Design review of the part shown in the three views and the two pictorial views. Dimensions are in mm from the part's minimum x, y and z. A direction names the side the tool comes from. Round coordinates to 2 decimals unless told otherwise and drop trailing zeros. Loops run counter-clockwise (first coordinate to the right, second up) from the corner with the lowest first, then second, coordinate; pieces in that order, holes last.
1) Take a section at B-B (y = 116). State the section outline as (x, z) points, then the cut area to 3 significant figures.
2) Wall thickness on L1, parallel to Y at x = 194.5, z = 701: over which ranges is the line inside the solid? List them lowest first.
3) Mouldability with a two-part tool opening along X and no side actions: class the marked faces 3, 4 and 5 as pulls with the +X half, pulls with the -X half, needs draft (parallel to the pull), parting line crosses it, or undercut.
4) Take a section at A-A (z = 564.5). State the section outline as (x, y) points.
5) Tool access review of the marked faces 1 and 2: name each direction out of +Z, -Z, +X, -X, +Y, -Y from which nothing blocks a thin tool from reaching the whole face with its end or side.
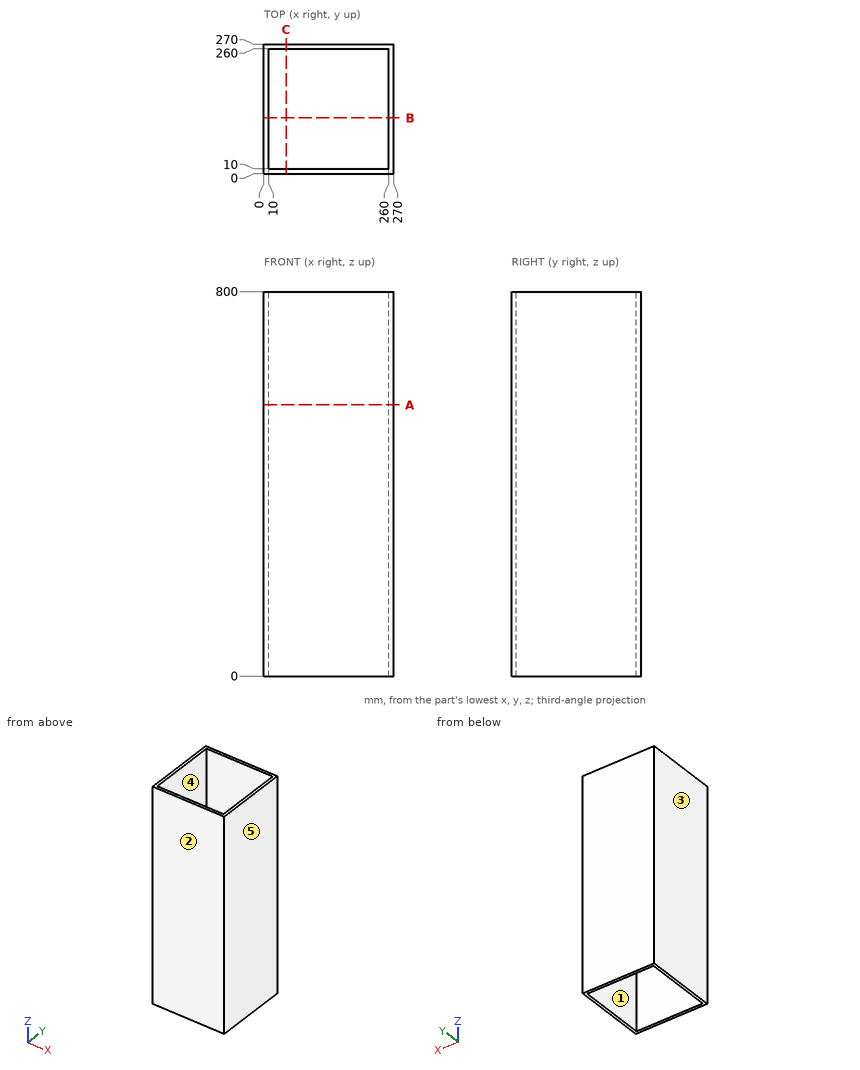
Response:
1. outline: (0, 0) - (10, 0) - (10, 800) - (0, 800) - close; (260, 0) - (270, 0) - (270, 800) - (260, 800) - close
1. area: 16,000 mm2
2. L1: y = 0 to 10, 260 to 270
3. face 3: pulls with the -X half
3. face 4: undercut
3. face 5: pulls with the +X half
4. outline: (0, 0) - (270, 0) - (270, 270) - (0, 270) - close; hole (10, 10) - (260, 10) - (260, 260) - (10, 260) - close
5. face 1: +Z, -Z
5. face 2: +Z, -Z, +X, -X, -Y
